Can you work these out from the model? Positions are in its coordinate system, mm. Round coordinates to 2 decimals unless told otherwise and drop trailing zeros. Order: outer loops, then holes, each group sorted by start corner. A loop starts at its lowest first (then second) coordinate and runs counter-clockwise, first axis right, second up. Notation, with made-up numbers: (58, 58) -> (112, 58) arc R30 cw to (112, 89) -> close; hole circle Ø2 at (-35, 21.5). An arc over 180 degrees is marked (long way). Use a Markdown table: item, result. Add a question column.
Q1. If we section it at A-A on z = -73: List the corners of the cut face in (x, y) for me, plus the area to 4 significant figures.
Q2. If we section it at C-C on y = -13.5: List the corners of the cut face in (x, z) for me.
Q3. I need wall thicknesses on line 1 along X through (y, z) = (-20.5, 122); line 2 along X through (y, z) = (-20, 59.5); line 3 along Y through (x, z) = (22.5, 27). Which ranges of each line are inside material? Lowest first, please. Write a range as [from, to].
Q4. I'm going to push flat-ended pins straight in: pin 1 Ø1 at (x, z) = (14, -27) entering from +Y; pin 2 Ø2 at (y, z) = (12.5, 4) entering from +X. Where does each tip first touch, or does it pass through?
Q5. If we section it at B-B on y = 12.5: List the corners of the cut face in (x, z) for me.
```python
from build123d import *

# Parameters (mm, degrees)
SKETCH1_W           = 280
SKETCH1_H           = 50
BOSS_EXTRUDE1_DEPTH = 25
CHAMFER1_SIZE       = 15


with BuildPart() as part:
    # Sketch1 → Boss-Extrude1 (new, symmetric)
    with BuildSketch(Plane(origin=(0, 0, 0), x_dir=(0, 0, -1), z_dir=(1, 0, 0))):
        Rectangle(SKETCH1_W, SKETCH1_H)
    extrude(amount=BOSS_EXTRUDE1_DEPTH, both=True)

    # Chamfer1
    chamfer1_edges = [part.edges().sort_by_distance(p)[0] for p in [
        (25, 25, 0),
        (25, -25, 0),
    ]]
    chamfer(chamfer1_edges, length=CHAMFER1_SIZE)


solid = part.part
```
Answer below:
| question | item | result |
|---|---|---|
| 1 | outline | (-25, -25) -> (10, -25) -> (25, -10) -> (25, 10) -> (10, 25) -> (-25, 25) -> close |
| 1 | area | 2,275 mm² |
| 2 | outline | (-25, -140) -> (21.5, -140) -> (21.5, 140) -> (-25, 140) -> close |
| 3 | line 1 | [-25, 14.5] |
| 3 | line 2 | [-25, 15] |
| 3 | line 3 | [-12.5, 12.5] |
| 4 | pin 1 | y = 21.5 |
| 4 | pin 2 | x = 23.5 |
| 5 | outline | (-25, -140) -> (22.5, -140) -> (22.5, 140) -> (-25, 140) -> close |
